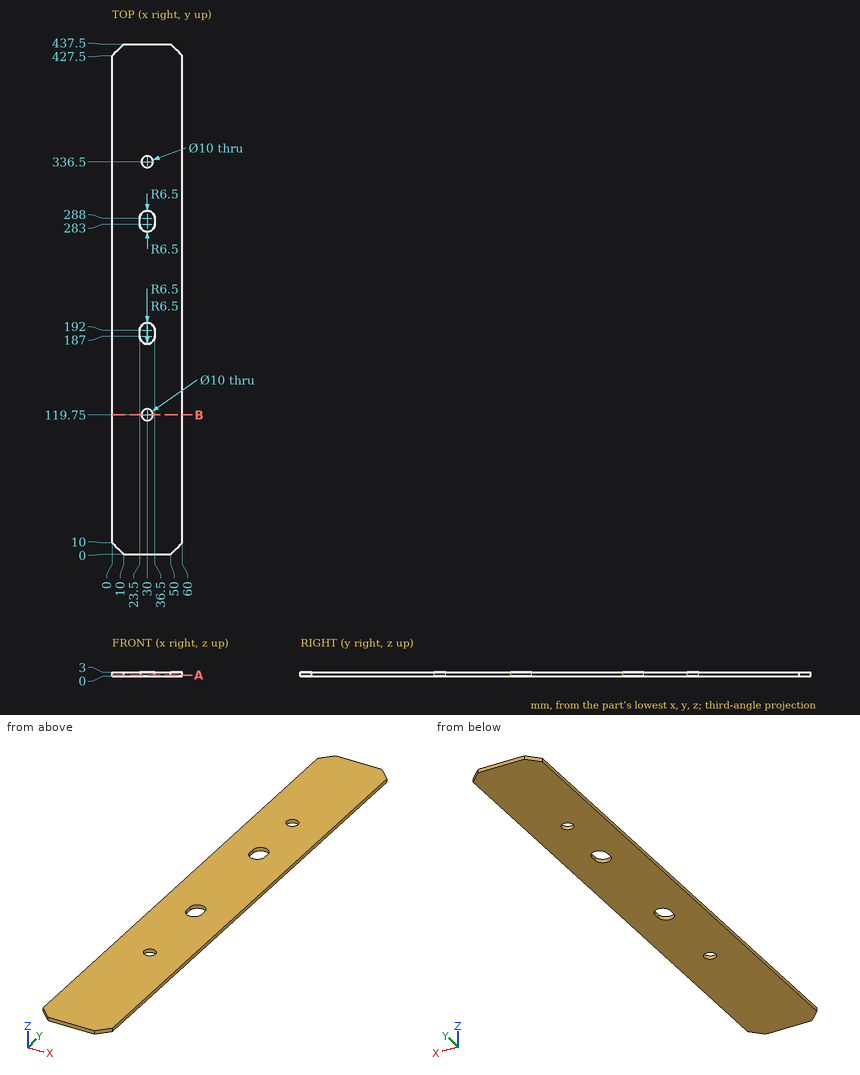
The figure shows three views and two pictorial views of one solid part (mm, origin at its lowest corner). Answer the questions. Give positions to 0.01 mm unless a question says otherwise; leave off trailing zeros. Write each loop counter-clockwise with the first axis right and the second up, starting at its lowest first coordinate (ties: lowest second). Pieces come first, ordered by that corner, then holes. Notation, with made-up numbers: (26, 78) -> (76, 78) arc R21 ccw to (76, 88) -> close; hole circle Ø3 at (64, 45.25). An arc over 180 degrees is marked (long way). Write each question's results on one line, items separated by ' | '.
1. Find section B-B on y = 119.75. Determine the outline of the cut face in (x, z).
Data:
outline: (0, 0) -> (25, 0) -> (25, 3) -> (0, 3) -> close; (35, 0) -> (60, 0) -> (60, 3) -> (35, 3) -> close
2. Straight lines are drawn through the part: L1, parallel to Y at x = 30, z = 1.05; L2, parallel to X at y = 190, z = 1.25; L3, parallel to Y at x = 25.5, z = 1.05. For each, find the intervals that lie inside material, in ascending order.
Data:
L1: 0 to 114.75, 124.75 to 180.5, 198.5 to 276.5, 294.5 to 331.5, 341.5 to 437.5 | L2: 0 to 23.5, 36.5 to 60 | L3: 0 to 117.57, 121.93 to 182.31, 196.69 to 278.31, 292.69 to 334.32, 338.68 to 437.5
3. Find section A-A on z = 0.65. Determine the outline of the cut face in (x, y), and give its area (3 significant figures).
Data:
outline: (0, 10) -> (10, 0) -> (50, 0) -> (60, 10) -> (60, 427.5) -> (50, 437.5) -> (10, 437.5) -> (0, 427.5) -> close; hole (23.5, 187) arc R6.5 ccw to (36.5, 187) -> (36.5, 192) arc R6.5 ccw to (23.5, 192) -> close; hole (23.5, 283) arc R6.5 ccw to (36.5, 283) -> (36.5, 288) arc R6.5 ccw to (23.5, 288) -> close; hole circle Ø10 at (30, 119.75); hole circle Ø10 at (30, 336.5) | area: 25,500 mm^2
